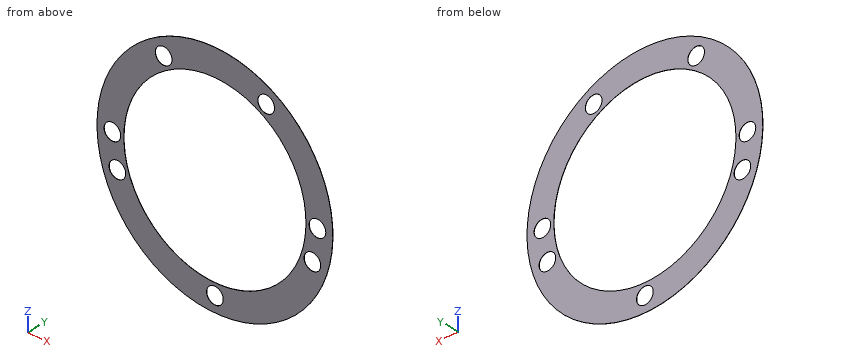
from build123d import *

# Parameters (mm, degrees)
SKETCH1_R                       = 146.05
SKETCH1_R_2                     = 112.776
BOSS_EXTRUDE1_DEPTH             = 0.254
F_13_16_0_8125_DIAMETER_HOLE1_D = 20.6375
F_13_16_0_8125_DIAMETER_HOLE2_D = 20.6375


with BuildPart() as part:
    # Sketch1 → Boss-Extrude1 (new body)
    with BuildSketch(Plane(origin=(0, 0, 0), x_dir=(1, 0, 0), z_dir=(0, 1, 0))):
        with Locations(Location((0, 0, 0), (0, 0, 270))):
            Circle(SKETCH1_R)
        with Locations(Location((0, 0, 0), (0, 0, 270))):
            Circle(SKETCH1_R_2, mode=Mode.SUBTRACT)
    extrude(amount=BOSS_EXTRUDE1_DEPTH)

    # 13/16 (0.8125) Diameter Hole1 (through all)
    with Locations(Plane(origin=(0, 0.254, 0), x_dir=(1, 0, 0), z_dir=(0, 1, 0))):
        with Locations((0, 127)):
            Hole(F_13_16_0_8125_DIAMETER_HOLE1_D / 2)

    # 13/16 (0.8125) Diameter Hole2 (through all)
    with Locations(Plane(origin=(0, 0, 0), x_dir=(-1, 0, 0), z_dir=(0, -1, 0))):
        with Locations((-63.5, -109.982), (-120.77, 39.243), (-127, 0)):
            f_13_16_0_8125_diameter_hole2 = Hole(F_13_16_0_8125_DIAMETER_HOLE2_D / 2)

    # Mirror1: 13/16 (0.8125) Diameter Hole2 across plane
    add(f_13_16_0_8125_diameter_hole2.mirror(Plane(origin=(0, 0, 0), x_dir=(0, 0, 1), z_dir=(1, 0, 0))), mode=Mode.SUBTRACT)


solid = part.part
Here's how the part is built. I have some questions about the finished solid (model axes, mm). Round coordinates to 2 decimals unless told otherwise and drop trailing zeros. Order: outer loops, then holes, each group sorted by start corner. A loop starts at its lowest first (then second) coordinate and runs counter-clockwise, first axis right, second up. Notation, with made-up numbers: (87.25, 0) -> (146.25, 0) arc R14 ccw to (146.25, 21) -> close; hole circle Ø8 at (-39, -13). An arc over 180 degrees is marked (long way). Return JSON: item names as keys, results as strings.
Q1. I need wall thicknesses on line 1 along Z through (x, y) = (-120.77, 0.1); line 2 along Z through (x, y) = (60, 0.1); line 3 along Z through (x, y) = (-47.5, 0.15). Which ranges of each line are inside material? Lowest first, please. Write a range as from..to.
Filled sheet:
{"line 1": "z = -82.13..-49.56, -28.92..-8.23, 8.23..82.13", "line 2": "z = -133.16..-95.49, 95.49..100.27, 119.69..133.16", "line 3": "z = -138.11..-102.28, 102.28..138.11"}
Q2. If we section it at B-B on x = 63.5: List the corners of the cut face in (y, z) for me, plus the area to 3 significant figures.
Filled sheet:
{"outline": "(0, -131.52) -> (0.25, -131.52) -> (0.25, -93.2) -> (0, -93.2) -> close; (0, 93.2) -> (0.25, 93.2) -> (0.25, 99.66) -> (0, 99.66) -> close; (0, 120.3) -> (0.25, 120.3) -> (0.25, 131.52) -> (0, 131.52) -> close", "area": "14.2 mm^2"}
Q3. If we section it at A-A on z = 0: List the corners of the cut face in (x, y) for me.
Filled sheet:
{"outline": "(-146.05, 0) -> (-137.32, 0) -> (-137.32, 0.25) -> (-146.05, 0.25) -> close; (-116.68, 0) -> (-112.78, 0) -> (-112.78, 0.25) -> (-116.68, 0.25) -> close; (112.78, 0) -> (116.68, 0) -> (116.68, 0.25) -> (112.78, 0.25) -> close; (137.32, 0) -> (146.05, 0) -> (146.05, 0.25) -> (137.32, 0.25) -> close"}
Q4. If we section it at C-C on x = 19: List the corners of the cut face in (y, z) for me.
Filled sheet:
{"outline": "(0, -144.81) -> (0.25, -144.81) -> (0.25, -111.16) -> (0, -111.16) -> close; (0, 111.16) -> (0.25, 111.16) -> (0.25, 144.81) -> (0, 144.81) -> close"}
Q5. If we section it at D-D on y = 0.15: Give the number of separate pieces and of enclosed holes in the cut face, plus the area to 3 significant figures.
Filled sheet:
{"separate pieces": "1", "enclosed holes": "8", "area": "24,700 mm^2"}
